from build123d import *

# Parameters (mm, degrees)
SKETCH1_W           = 85
SKETCH1_H           = 120
SKETCH1_R           = 5.5
SKETCH1_W_2         = 40
SKETCH1_H_2         = 40
BOSS_EXTRUDE1_DEPTH = 20
SKETCH2_R           = 10.75
CUT_EXTRUDE1_DEPTH  = 15
SKETCH3_R           = 3
CUT_EXTRUDE2_DEPTH  = 106.948100502


with BuildPart() as part:
    # Sketch1 → Boss-Extrude1 (new body)
    with BuildSketch(Plane(origin=(0, 0, 0), x_dir=(1, 0, 0), z_dir=(0, 1, 0))):
        Rectangle(SKETCH1_W, SKETCH1_H)
        with Locations(Location((-30, 40, 0), (0, 0, 270))):
            Circle(SKETCH1_R, mode=Mode.SUBTRACT)
        with Locations(Location((30, 40, 0), (0, 0, 270))):
            Circle(SKETCH1_R, mode=Mode.SUBTRACT)
        with Locations(Location((30, -40, 0), (0, 0, 270))):
            Circle(SKETCH1_R, mode=Mode.SUBTRACT)
        with Locations(Location((-30, -40, 0), (0, 0, 270))):
            Circle(SKETCH1_R, mode=Mode.SUBTRACT)
        with Locations((7.5, 0)):
            Rectangle(SKETCH1_W_2, SKETCH1_H_2, mode=Mode.SUBTRACT)
    extrude(amount=BOSS_EXTRUDE1_DEPTH)

    # Sketch2 → Cut-Extrude1 (cut)
    with BuildSketch(Plane(origin=(0, 20, 0), x_dir=(1, 0, 0), z_dir=(0, 1, 0))):
        with Locations(Location((30, 40, 0), (0, 0, 270))):
            Circle(SKETCH2_R)
        with Locations(Location((-30, 40, 0), (0, 0, 270))):
            Circle(SKETCH2_R)
        with Locations(Location((-30, -40, 0), (0, 0, 270))):
            Circle(SKETCH2_R)
        with Locations(Location((30, -40, 0), (0, 0, 270))):
            Circle(SKETCH2_R)
    extrude(amount=-CUT_EXTRUDE1_DEPTH, mode=Mode.SUBTRACT)

    # Sketch3 → Cut-Extrude2 (cut, through all)
    with BuildSketch(Plane.ZY.offset(42.5)):
        with Locations((0, 10)):
            Circle(SKETCH3_R)
    extrude(amount=-CUT_EXTRUDE2_DEPTH, mode=Mode.SUBTRACT)


solid = part.part
Verification items for the finished model (mm, model axes). A direction names the side the tool comes from. Coordinates: 2 decimals unless noted, no trailing zeros. Order: outer loops, then holes, each group sorted by start corner. A loop starts at its lowest first (then second) coordinate and runs counter-clockwise, first axis right, second up. Notation, with made-up numbers: M -29,52.25 L -8,52.25 A15 cw -8,56.25 Z; hole C 82,86 d6. An arc over 180 degrees is marked long. Return JSON: item names as keys, results as strings.
1) Cross-section at C-C, the plane z = -40. Record the boundary of the cut face in (x, y).
Answer list:
{"outline": "M -42.5,0 L -35.5,0 L -35.5,5 L -40.75,5 L -40.75,20 L -42.5,20 Z; M -24.5,0 L 24.5,0 L 24.5,5 L 19.25,5 L 19.25,20 L -19.25,20 L -19.25,5 L -24.5,5 Z; M 35.5,0 L 42.5,0 L 42.5,20 L 40.75,20 L 40.75,5 L 35.5,5 Z"}
2) Thickness scan on L1, parallel to Z at x = -30, y = 3.6; L2, parallel to X at y = 2, z = 40; L3, parallel to X at y = 9.75, z = 5.5. Record the ranges inside material, lowest first. Write a range as [from, to].
Answer list:
{"L1": "[-60, -45.5], [-34.5, 34.5], [45.5, 60]", "L2": "[-42.5, -35.5], [-24.5, 24.5], [35.5, 42.5]", "L3": "[-42.5, -12.5], [27.5, 42.5]"}
3) Gauge pin test, flat end, axial feed: pin 1 (11 mm diameter, centred on x = -33.5, z = 44, fed in from +Y). Record the tip position at first contact, or that the pin passes through.
Answer list:
{"pin 1": "y = 20"}
4) Cross-section at D-D, the plane y = 15.5. Record the boundary of the cut face in (x, z), and give its area (3 significant figures).
Answer list:
{"outline": "M -42.5,-60 L 42.5,-60 L 42.5,60 L -42.5,60 Z; hole C -30,-40 d21.5; hole C -30,40 d21.5; hole M -12.5,-20 L 27.5,-20 L 27.5,20 L -12.5,20 Z; hole C 30,-40 d21.5; hole C 30,40 d21.5", "area": "7,150 mm2"}
5) Cross-section at A-A, the plane y = 10. Record the boundary of the cut face in (x, z), and give its area (3 significant figures).
Answer list:
{"outline": "M -42.5,-60 L 42.5,-60 L 42.5,-3 L 27.5,-3 L 27.5,-20 L -12.5,-20 L -12.5,-3 L -42.5,-3 Z; M -42.5,3 L -12.5,3 L -12.5,20 L 27.5,20 L 27.5,3 L 42.5,3 L 42.5,60 L -42.5,60 Z; hole C -30,-40 d21.5; hole C -30,40 d21.5; hole C 30,-40 d21.5; hole C 30,40 d21.5", "area": "6,880 mm2"}
6) Release check for a two-part mould opening along Z. For faces 1 (the flat face through (35, 5, -43)), 2 (the flat face through (-1, 10, 60)), 3 (the flat face through (-42.5, 5, 1)) record: +Z half, -Z half, draft (parallel to the pull), parting line (faces both ways), or undercut.
Answer list:
{"face 1": "undercut", "face 2": "+Z half", "face 3": "draft"}
7) Cross-section at B-B, the plane x = 30. Record the boundary of the cut face in (y, z), and give its area (3 significant figures).
Answer list:
{"outline": "M 0,-60 L 20,-60 L 20,-50.75 L 5,-50.75 L 5,-45.5 L 0,-45.5 Z; M 0,-34.5 L 5,-34.5 L 5,-29.25 L 20,-29.25 L 20,29.25 L 5,29.25 L 5,34.5 L 0,34.5 Z; M 0,45.5 L 5,45.5 L 5,50.75 L 20,50.75 L 20,60 L 0,60 Z; hole C 10,0 d6", "area": "1,620 mm2"}
8) Access from +Z, -Z, +X, -X, +Y, -Y to the whole of each face (thin tool, end or side, straight path). Record for faces 4 (the cylindrical face through (33.229, 12.605, -29.746)), 5 (the flat face through (27.5, 5, 0)), 6 (the flat face through (-19, 0, -1)).
Answer list:
{"face 4": "+Y", "face 5": "+Y, -Y", "face 6": "+Z, -Z, +X, -X, -Y"}
